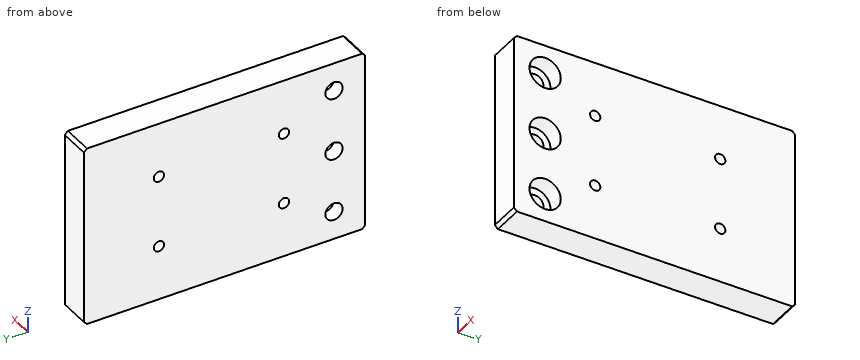
from build123d import *

# Parameters (mm, degrees)
SKETCH_1_W                   = 58
SKETCH_1_H                   = 90
EXTRUDE_1_DEPTH              = 10
HOLE_WIZARD_M4_1_D           = 3.3
HOLE_WIZARD_M5_1_D           = 5.5
HOLE_WIZARD_M5_1_CBORE_D     = 10
HOLE_WIZARD_M5_1_CBORE_DEPTH = 5.4
CHAMFER_1_SIZE               = 1


with BuildPart() as part:
    # 草图1 → 凸台-拉伸1 (new body)
    with BuildSketch(Plane(origin=(0, 0, 0), x_dir=(0, 0, -1), z_dir=(1, 0, 0))):
        Rectangle(SKETCH_1_W, SKETCH_1_H)
    extrude(amount=EXTRUDE_1_DEPTH)

    # M4 螺纹孔1 (through all)
    with Locations(Plane(origin=(10, 0, 0), x_dir=(0, 0, -1), z_dir=(1, 0, 0))):
        with Locations((-11.5, 21), (11.5, 21), (-11.5, -19), (11.5, -19)):
            Hole(HOLE_WIZARD_M4_1_D / 2)

    # M5 六角凹头螺钉的柱形沉头孔1 (through all)
    with Locations(Plane(origin=(10, 0, 0), x_dir=(0, 0, -1), z_dir=(1, 0, 0))):
        with Locations((-20, -35), (0, -35), (20, -35)):
            CounterBoreHole(HOLE_WIZARD_M5_1_D / 2, HOLE_WIZARD_M5_1_CBORE_D / 2, HOLE_WIZARD_M5_1_CBORE_DEPTH)

    # 倒角1
    chamfer_1_edges = [part.edges().sort_by_distance(p)[0] for p in [
        (5, -45, -29),
        (5, -45, 29),
        (5, 45, 29),
        (5, 45, -29),
    ]]
    chamfer(chamfer_1_edges, length=CHAMFER_1_SIZE)


solid = part.part
Input: part model. Units: mm. Frame: model coordinates. Coordinates: 2 decimals unless noted, no trailing zeros. Loops run counter-clockwise (first coordinate to the right, second up) from the corner with the lowest first, then second, coordinate; pieces in that order, holes last. Notation, with made-up numbers: (70, -25) -> (88, -25) arc R11 cw to (88, -9) -> close; hole circle Ø5 at (36.5, 24). An arc over 180 degrees is marked (long way). One line per item, written item: value.
(1) Pin query (flat end, axial travel): pin 1 Ø3 at (y, z) = (-37.5, -21) entering from +X. Return the tip coordinate at first contact, or that it passes through.
Answer below:
pin 1: stops at x = 4.6
(2) Cut plane C-C (x = 2.5). Output: boundary loops of the cut face in (y, z).
Answer below:
outline: (-45, -28) -> (-44, -29) -> (44, -29) -> (45, -28) -> (45, 28) -> (44, 29) -> (-44, 29) -> (-45, 28) -> close; hole circle Ø5.5 at (-35, -20); hole circle Ø5.5 at (-35, 0); hole circle Ø5.5 at (-35, 20); hole circle Ø3.3 at (-19, -11.5); hole circle Ø3.3 at (-19, 11.5); hole circle Ø3.3 at (21, -11.5); hole circle Ø3.3 at (21, 11.5)
(3) Cut plane B-B (y = 21). Output: boundary loops of the cut face in (x, z).
Answer below:
outline: (0, -29) -> (10, -29) -> (10, -13.15) -> (0, -13.15) -> close; (0, -9.85) -> (10, -9.85) -> (10, 9.85) -> (0, 9.85) -> close; (0, 13.15) -> (10, 13.15) -> (10, 29) -> (0, 29) -> close
(4) Ray query, line 1 along Y through (x, z) = (7.8, -20); line 2 along Y through (x, z) = (1.1, 0); line 3 along Z through (x, y) = (1.5, -19.5). Return the intervals inside material, ascending.
Answer below:
line 1: y = -45 to -40, -30 to 45
line 2: y = -45 to -37.75, -32.25 to 45
line 3: z = -29 to -13.07, -9.93 to 9.93, 13.07 to 29
(5) Cut plane A-A (z = -20). Output: boundary loops of the cut face in (x, y), then the cut area to 3 significant figures.
Answer below:
outline: (0, -45) -> (10, -45) -> (10, -40) -> (4.6, -40) -> (4.6, -37.75) -> (0, -37.75) -> close; (0, -32.25) -> (4.6, -32.25) -> (4.6, -30) -> (10, -30) -> (10, 45) -> (0, 45) -> close
area: 821 mm2
(6) Cut plane D-D (z = 11.5). Output: boundary loops of the cut face in (x, y).
Answer below:
outline: (0, -45) -> (10, -45) -> (10, -20.65) -> (0, -20.65) -> close; (0, -17.35) -> (10, -17.35) -> (10, 19.35) -> (0, 19.35) -> close; (0, 22.65) -> (10, 22.65) -> (10, 45) -> (0, 45) -> close
